Geometry check sheet. Reference: the model listing, model coordinates, mm. A direction names the side the tool comes from. Round coordinates to 2 decimals unless told otherwise and drop trailing zeros. Order: outer loops, then holes, each group sorted by start corner. A loop starts at its lowest first (then second) coordinate and runs counter-clockwise, first axis right, second up. Notation, with made-up numbers: (-30.75, 42.5) - (-17.75, 42.5) arc R25 cw to (-17.75, 65.5) - close; hole circle Ø11 at (70.25, 75.5). An arc over 180 degrees is marked (long way). Return JSON: item names as keys, results as strings. Group by question number.
Q1. Sectioned sample at B-B, the plane z = 46. Record the cut outline in (x, y), then the cut area to 3 significant figures.
Q2. Sectioned sample at A-A, the plane y = -33. Record the cut outline in (x, z), then the cut area to 3 significant figures.
Q3. Sectioned sample at D-D, the plane y = 27.5. Record the cut outline in (x, z).
Q4. Gauge pin test, flat ends, axial feed: pin 1 Ø8 at (x, z) = (41, 28.5) entering from +Y; pin 2 Ø4 at (x, y) = (-125.5, -50.5) entering from +Z; pin 3 Ø2 at (x, y) = (-23.5, 25) entering from +Z. Record the tip position at first contact, or that the pin passes through.
Q5. Sectioned sample at C-C, the plane x = 104. Record the cut outline in (y, z).
Q6. Material ranges on line 1 along X through (y, z) = (-24, 185); line 2 along Y through (x, z) = (-83, 79); line 3 along Y through (x, z) = (97, -234), recorded low to high.
Q7. Tool access check on faces 1 (the cylindrical face through (9.893, 4.93, -224.782)), 2 (the cylindrical face through (-20.6, 27.79, -26.86)), 3 (the flat face through (0, 43, 0)). Record the directions out of +Z, -Z, +X, -X, +Y, -Y that give a thin tool (end or side, any length) a straight path to the whole face; none if there is none.
```python
from build123d import *

# Parameters (mm, degrees)
SKETCH1_R           = 225
BOSS_EXTRUDE2_DEPTH = 10
SKETCH2_R           = 5
BOSS_EXTRUDE3_DEPTH = 100
SKETCH3_R           = 255
BOSS_EXTRUDE5_DEPTH = 3
SKETCH7_R           = 33.849496271
BOSS_EXTRUDE6_DEPTH = 30


with BuildPart() as part:
    # Sketch1 → Boss-Extrude2 (new body)
    with BuildSketch(Plane(origin=(0, 0, 0), x_dir=(1, 0, 0), z_dir=(0, 1, 0))):
        with Locations(Location((0, 0, 0), (0, 0, 270))):
            Circle(SKETCH1_R)
    extrude(amount=BOSS_EXTRUDE2_DEPTH)

    # Sketch2 → Boss-Extrude3 (add)
    with BuildSketch(Plane.XZ):
        with Locations(Location((-185, 0, 0), (0, 0, 90))):
            Circle(SKETCH2_R)
        with Locations(Location((-130.81475452, 130.81475452, 0), (0, 0, 90))):
            Circle(SKETCH2_R)
        with Locations(Location((0, 185, 0), (0, 0, 90))):
            Circle(SKETCH2_R)
        with Locations(Location((130.81475452, 130.81475452, 0), (0, 0, 90))):
            Circle(SKETCH2_R)
        with Locations(Location((185, 0, 0), (0, 0, 90))):
            Circle(SKETCH2_R)
        with Locations(Location((130.81475452, -130.81475452, 0), (0, 0, 90))):
            Circle(SKETCH2_R)
        with Locations(Location((0, -185, 0), (0, 0, 90))):
            Circle(SKETCH2_R)
        with Locations(Location((-130.81475452, -130.81475452, 0), (0, 0, 90))):
            Circle(SKETCH2_R)
    extrude(amount=BOSS_EXTRUDE3_DEPTH)

    # Sketch3 → Boss-Extrude5 (add)
    with BuildSketch(Plane(origin=(0, 10, 0), x_dir=(1, 0, 0), z_dir=(0, 1, 0))):
        with Locations(Location((0, 0, 0), (0, 0, 270))):
            Circle(SKETCH3_R)
    extrude(amount=BOSS_EXTRUDE5_DEPTH)

    # Sketch7 → Boss-Extrude6 (add)
    with BuildSketch(Plane(origin=(0, 13, 0), x_dir=(1, 0, 0), z_dir=(0, 1, 0))):
        with Locations(Location((0, 0, 0), (0, 0, 270))):
            Circle(SKETCH7_R)
    extrude(amount=BOSS_EXTRUDE6_DEPTH)


solid = part.part
```
Reply:
{
 "1": {"outline": "(-250.82, 10) - (-220.25, 10) - (-220.25, 0) - (220.25, 0) - (220.25, 10) - (250.82, 10) - (250.82, 13) - (-250.82, 13) - close", "area": "5,910 mm^2"},
 "2": {"outline": "circle Ø10 at (-185, 0); circle Ø10 at (-130.81, -130.81); circle Ø10 at (-130.81, 130.81); circle Ø10 at (0, -185); circle Ø10 at (0, 185); circle Ø10 at (130.81, -130.81); circle Ø10 at (130.81, 130.81); circle Ø10 at (185, 0)", "area": "628 mm^2"},
 "3": {"outline": "circle Ø67.7 at (0, 0)"},
 "4": {"pin 1": "y = 13", "pin 2": "z = 134.56", "pin 3": "z = 25.29"},
 "5": {"outline": "(0, -199.52) - (10, -199.52) - (10, -232.83) - (13, -232.83) - (13, 232.83) - (10, 232.83) - (10, 199.52) - (0, 199.52) - close"},
 "6": {"line 1": "-5 to 5", "line 2": "0 to 13", "line 3": "10 to 13"},
 "7": {"face 1": "-Y", "face 2": "+Y", "face 3": "+Z, -Z, +X, -X, +Y"}
}
